```python
from build123d import *

# Parameters (mm, degrees)
BRACKET_PROFILE_SKETCH_R   = 7.5
BRACKET_PROFILE_BOSS_DEPTH = 20
BASE_BLOCK_SKETCH_R        = 10
BASE_BLOCK_BOSS_DEPTH      = 20


with BuildPart() as part:
    # Bracket Profile Sketch → Bracket Profile Boss (new body)
    with BuildSketch(Plane(origin=(0, 0, 0), x_dir=(0, 0, -1), z_dir=(1, 0, 0))):
        with BuildLine():
            Line((55, 0), (55, -15))
            Line((55, -15), (-55.001498604, -15))
            Line((-55.001498604, -15), (-55, 0))
            ThreePointArc((-55, 0), (-50.606601718, 10.606601718), (-40, 15))
            ThreePointArc((-40, 15), (-24.521101379, 30.372215271), (-15, 50))
            ThreePointArc((-15, 50), (0, 65), (15, 50))
            ThreePointArc((15, 50), (24.521101379, 30.372215271), (40, 15))
            ThreePointArc((40, 15), (50.606601718, 10.606601718), (55, 0))
        make_face()
        with Locations((0, 50)):
            Circle(BRACKET_PROFILE_SKETCH_R, mode=Mode.SUBTRACT)
        with Locations((40, 0)):
            Circle(BRACKET_PROFILE_SKETCH_R, mode=Mode.SUBTRACT)
        with Locations((-40, 0)):
            Circle(BRACKET_PROFILE_SKETCH_R, mode=Mode.SUBTRACT)
    extrude(amount=BRACKET_PROFILE_BOSS_DEPTH)

    # Base Block Sketch → Base Block Boss (add)
    with BuildSketch(Plane(origin=(0, -15, 0), x_dir=(-1, 0, 0), z_dir=(0, -1, 0))):
        with BuildLine():
            Line((-20, 55), (-20, -55.001498604))
            Line((-20, -55.001498604), (0, -55.001498604))
            Line((0, -55.001498604), (40, -55.001498604))
            ThreePointArc((40, -55.001498604), (57.794589541, -44.131262187), (56.246039556, -23.336756912))
            Line((56.246039556, -23.336756912), (0, 55))
            Line((0, 55), (-20, 55))
        make_face()
        with Locations(Location((40, -35.001498604, 0), (0, 0, 90))):
            Circle(BASE_BLOCK_SKETCH_R, mode=Mode.SUBTRACT)
    extrude(amount=BASE_BLOCK_BOSS_DEPTH)


solid = part.part
```
Input: part model. Units: mm. Frame: model coordinates. A direction names the side the tool comes from. Give positions to 0.01 mm unless a question says otherwise; leave off trailing zeros. Order: outer loops, then holes, each group sorted by start corner. A loop starts at its lowest first (then second) coordinate and runs counter-clockwise, first axis right, second up.
1. Section C-C on y = -27.5. Return the cut outline in (x, z), and give its area (3 significant figures).
Derived:
outline: (-56.25, 23.34) - (0, -55) - (20, -55) - (20, 55) - (-40, 55) arc R20 ccw to start; hole circle Ø20 at (-40, 35)
area: 5,890 mm2
2. Section B-B on x = 8. Return the cut outline in (y, z).
Derived:
outline: (-35, -55) - (0, -55) arc R15 ccw to (15, -40) arc R65 cw to (50, -15) arc R15 ccw to (50, 15) arc R65 cw to (15, 40) arc R15 ccw to (0, 55) - (-15, 55) - (-35, 55) - close; hole circle Ø15 at (0, -40); hole circle Ø15 at (0, 40); hole circle Ø15 at (50, 0)
3. Mould query, pull axis X, two halves, no side actions, for faces 3 (the flat face through (10, -17, -55)), 4 (the cylindrical face through (-46, -25, 43)), 5 (the flat face through (20, 5, -1)), 6 (the flat face through (-28.52, -24.86, -15.28)). Classes: released by +X, released by -X, zero draft, split by the parting line, or undercut.
Derived:
face 3: zero draft
face 4: undercut
face 5: released by +X
face 6: released by -X
4. Pin query (flat end, axial travel): pin 1 (1.5 mm diameter, centred on x = -8, z = 1, fed in from +Y). Return the tip coordinate at first contact, or that it passes through.
Derived:
pin 1: stops at y = -15
5. Reachability of faces 1 (the cylindrical face through (9.86, 10.72, -50.49)), 2 (the flat face through (-23, -15, 11)) from +Z, -Z, +X, -X, +Y, -Y: full face, straight path, thin tool, end or side. Return the list, or none.
Derived:
face 1: -Z, +X, -X, +Y
face 2: +Z, -Z, -X, +Y
6. Section D-D on z = 0. Return the cut outline in (x, y).
Derived:
outline: (-39.49, -35) - (20, -35) - (20, 42.5) - (0, 42.5) - (0, -15) - (-39.49, -15) - close; (0, 57.5) - (20, 57.5) - (20, 65) - (0, 65) - close
7. Material intervals for L1, parallel to Y at x = 6.75, z = 0; L2, parallel to Y at x = 10.75, z = 40; L3, parallel to Y at x = -8.5, z = 12.5, sorted ascending.
Derived:
L1: y = -35 to 42.5, 57.5 to 65
L2: y = -35 to -7.5, 7.5 to 15
L3: y = -35 to -15
8. Section A-A on z = 42. Return the cut outline in (x, y).
Derived:
outline: (-58.74, -35) - (-47.14, -35) - (-47.14, -15) - (-58.74, -15) - close; (-32.86, -35) - (20, -35) - (20, -7.23) - (0, -7.23) - (0, -15) - (-32.86, -15) - close; (0, 7.23) - (20, 7.23) - (20, 14.87) - (0, 14.87) - close
